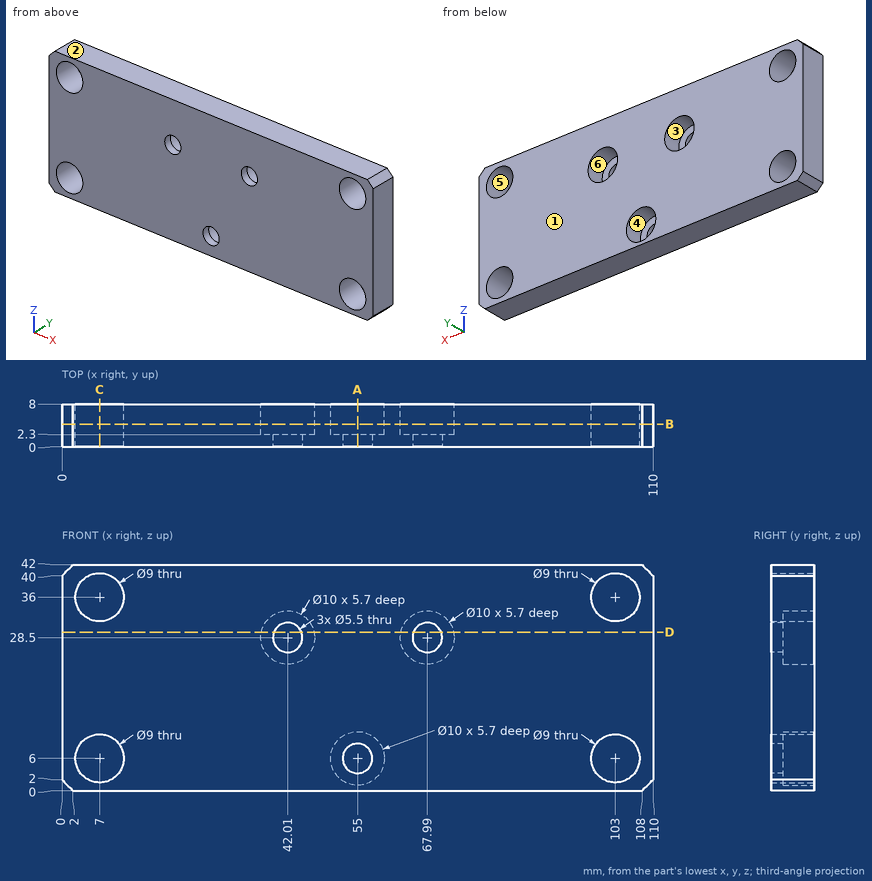
Study the drawing (mm; zero at the part's minimum x, y, z) and answer. A direction names the side the tool comes from. Coordinates: 2 decimals unless noted, no trailing zeros. Write each loop counter-clockwise with the first axis right and the second up, starting at its lowest first coordinate (ties: lowest second). Pieces come first, ordered by that corner, then holes. Notation, with made-up numbers: (14.25, -35) -> (73.25, -35) arc R22 cw to (73.25, -7) -> close; hole circle Ø11 at (-18, 7.25). An arc over 180 degrees is marked (long way). Write item = value, one per line.
(1) Section B-B on y = 4.25 is taken. Write down the section's boundary in (x, z).
From the geometry:
outline = (0, 2) -> (2, 0) -> (108, 0) -> (110, 2) -> (110, 40) -> (108, 42) -> (2, 42) -> (0, 40) -> close; hole circle Ø9 at (7, 6); hole circle Ø9 at (7, 36); hole circle Ø10 at (42.01, 28.5); hole circle Ø10 at (55, 6); hole circle Ø10 at (67.99, 28.5); hole circle Ø9 at (103, 6); hole circle Ø9 at (103, 36)
(2) Given pin 1 Ø5 at (x, z) = (55, 7) entering from +Y, flat-ended and moving along its own axis, determine where the tip first touches the part or whether it passes through.
From the geometry:
pin_1 = 2.3
(3) Section D-D on z = 29.5 is taken. Write down the section's boundary in (x, y).
From the geometry:
outline = (0, 0) -> (39.45, 0) -> (39.45, 2.3) -> (37.11, 2.3) -> (37.11, 8) -> (0, 8) -> close; (44.57, 0) -> (65.43, 0) -> (65.43, 2.3) -> (63.09, 2.3) -> (63.09, 8) -> (46.91, 8) -> (46.91, 2.3) -> (44.57, 2.3) -> close; (70.55, 0) -> (110, 0) -> (110, 8) -> (72.89, 8) -> (72.89, 2.3) -> (70.55, 2.3) -> close
(4) Section C-C on x = 7 is taken. Write down the section's boundary in (y, z), plus the area to 3 significant figures.
From the geometry:
outline = (0, 0) -> (8, 0) -> (8, 1.5) -> (0, 1.5) -> close; (0, 10.5) -> (8, 10.5) -> (8, 31.5) -> (0, 31.5) -> close; (0, 40.5) -> (8, 40.5) -> (8, 42) -> (0, 42) -> close
area = 192 mm2
(5) Straight lines are drawn through the part: L1, parallel to Z at x = 103, y = 2.5; L2, parallel to X at y = 5.7, z = 28.5; L3, parallel to Z at x = 55, y = 1.05. For each, find the intervals that lie inside material, in ascending order. Write a range as from..to.
From the geometry:
L1 = 0..1.5, 10.5..31.5, 40.5..42
L2 = 0..37.01, 47.01..62.99, 72.99..110
L3 = 0..3.25, 8.75..42
(6) For a pull along Z with two mould halves and no side action, classify the marked faces 1, 2, 3 and 4 as +Z half, -Z half, draft (parallel to the pull), parting line (faces both ways), or undercut.
From the geometry:
face_1 = draft
face_2 = +Z half
face_3 = undercut
face_4 = undercut
(7) Section A-A on x = 55 is taken. Write down the section's boundary in (y, z).
From the geometry:
outline = (0, 0) -> (8, 0) -> (8, 1) -> (2.3, 1) -> (2.3, 3.25) -> (0, 3.25) -> close; (0, 8.75) -> (2.3, 8.75) -> (2.3, 11) -> (8, 11) -> (8, 42) -> (0, 42) -> close
(8) Which of the six approach directions +Z, -Z, +X, -X, +Y, -Y give full straight-line access (tool end or side, diameter ignored) to the marked faces 5 and 6?
From the geometry:
face_5 = +Y, -Y
face_6 = +Y
